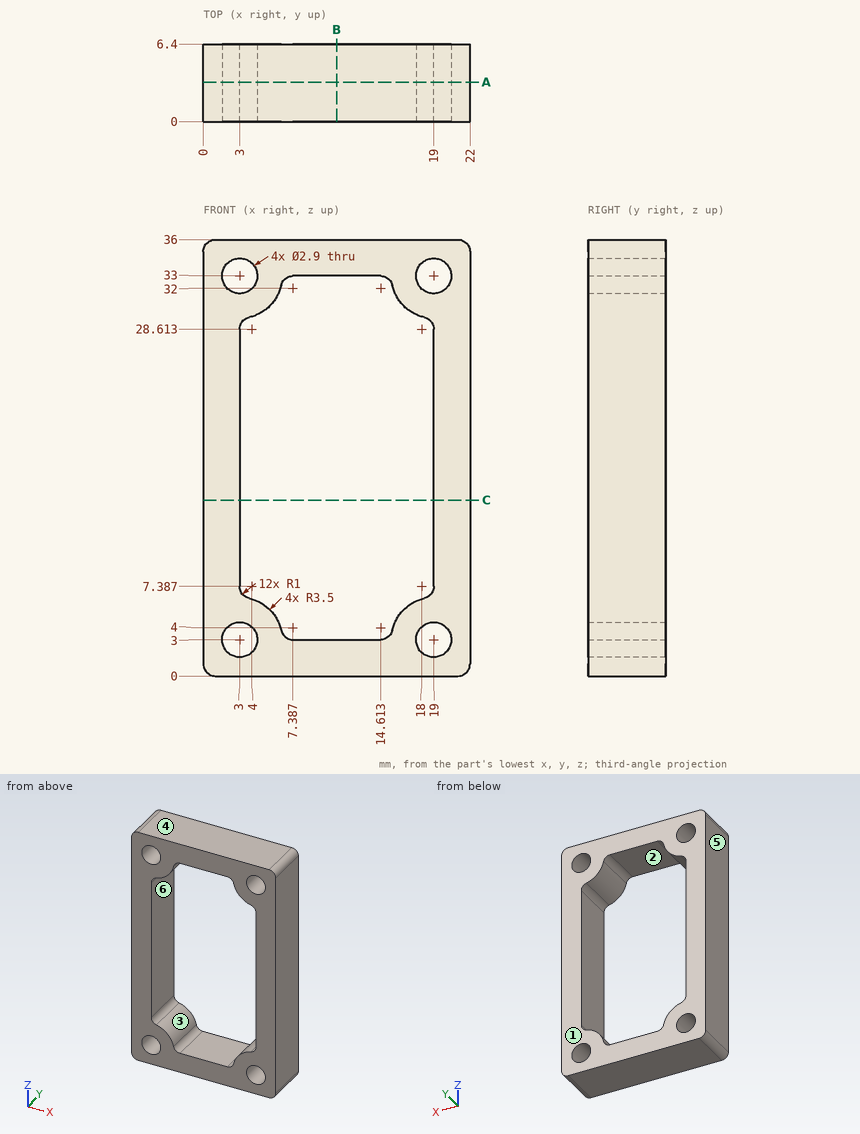
Input: dimensioned drawing with shaded views. Units: mm. Origin: part minimum x, y, z. A direction names the side the tool comes from. Coordinates: 2 decimals unless noted, no trailing zeros. Loops run counter-clockwise (first coordinate to the right, second up) from the corner with the lowest first, then second, coordinate; pieces in that order, holes last. Notation, with made-up numbers: M 23.25,-2.75 L 62.25,-2.75 A8 ccw 62.25,10.25 Z; hole C -40,-5 d11. An arc over 180 degrees is marked long. One line per item, written item: value. Start each with the question number.
1) Reachability of the marked faces 5 and 6 from +Z, -Z, +X, -X, +Y, -Y: full face, straight path, thin tool, end or side. Return the list, or none.
2) Cut plane C-C (z = 14.5). Return loops of the section in (x, y).
3) Cut plane A-A (y = 3.25). Return loops of the section in (x, z).
4) Draft query along Z for the marked faces 1, 2, 3 and 4. Return one class per face: released by +Z, released by -Z, zero draft, split by the parting line, or undercut.
5) Cut plane B-B (x = 11). Return loops of the section in (y, z), then the cut area to 3 significant figures.
6) Material intervals for L1, parallel to Z at x = 9.75, y = 5.25; L2, parallel to X at y = 3.5, z = 16.5; L3, parallel to Z at x = 3.75, y = 4.5, sorted ascending. Write a range as from..to.
Evaluation:
1. face 5: +Z, -Z, -X, +Y, -Y
1. face 6: +Y, -Y
2. outline: M 0,0 L 3,0 L 3,6.4 L 0,6.4 Z; M 19,0 L 22,0 L 22,6.4 L 19,6.4 Z
3. outline: M 0,1 A1 ccw 1,0 L 21,0 A1 ccw 22,1 L 22,35 A1 ccw 21,36 L 1,36 A1 ccw 0,35 Z; hole C 3,3 d2.9; hole C 3,33 d2.9; hole M 3,7.39 A1 ccw 3.78,6.41 A3.5 cw 6.41,3.78 A1 ccw 7.39,3 L 14.61,3 A1 ccw 15.59,3.78 A3.5 cw 18.22,6.41 A1 ccw 19,7.39 L 19,28.61 A1 ccw 18.22,29.59 A3.5 cw 15.59,32.22 A1 ccw 14.61,33 L 7.39,33 A1 ccw 6.41,32.22 A3.5 cw 3.78,29.59 A1 ccw 3,28.61 Z; hole C 19,3 d2.9; hole C 19,33 d2.9
4. face 1: zero draft
4. face 2: undercut
4. face 3: undercut
4. face 4: released by +Z
5. outline: M 0,0 L 6.4,0 L 6.4,3 L 0,3 Z; M 0,33 L 6.4,33 L 6.4,36 L 0,36 Z
5. area: 38.4 mm^2
6. L1: 0..3, 33..36
6. L2: 0..3, 19..22
6. L3: 0..1.76, 4.24..6.42, 29.58..31.76, 34.24..36
